Could you check a few things on this drawing? It's one solid part, dimensions in mm from its lowest x, y, z. A direction names the side the tool comes from. Coordinates: 2 decimals unless noted, no trailing zeros. Write each loop counter-clockwise with the first axis right and the second up, starting at its lowest first coordinate (ties: lowest second). Pieces come first, ordered by that corner, then holes.
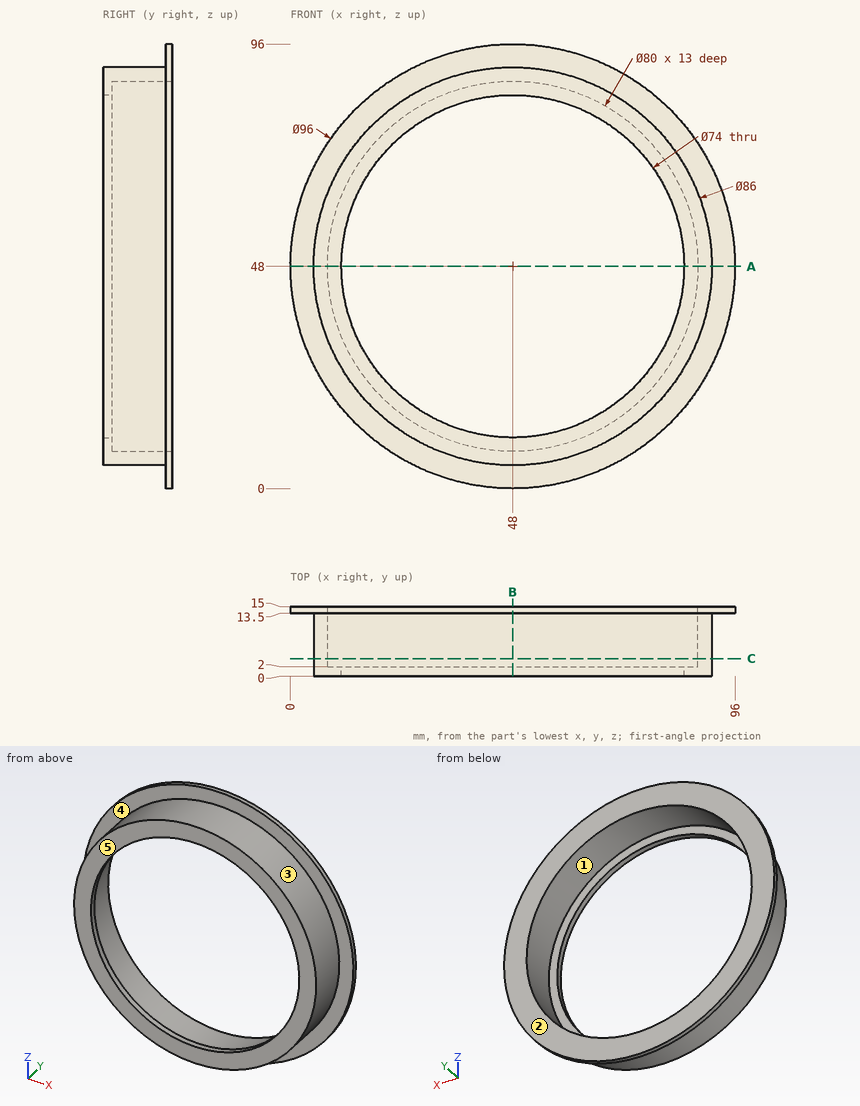
1) Imagine slicing it at B-B on x = 48. Please give me the cut outline in (y, z), then the cut area to 3 significant figures.
Values follow:
outline: (0, 5) - (13.5, 5) - (13.5, 0) - (15, 0) - (15, 8) - (2, 8) - (2, 11) - (0, 11) - close; (0, 85) - (2, 85) - (2, 88) - (15, 88) - (15, 96) - (13.5, 96) - (13.5, 91) - (0, 91) - close
area: 117 mm2
2) Imagine slicing it at A-A on z = 48. Please give me the cut outline in (x, y), then the cut area to 3 significant figures.
Values follow:
outline: (0, 13.5) - (5, 13.5) - (5, 0) - (11, 0) - (11, 2) - (8, 2) - (8, 15) - (0, 15) - close; (85, 0) - (91, 0) - (91, 13.5) - (96, 13.5) - (96, 15) - (88, 15) - (88, 2) - (85, 2) - close
area: 117 mm2
3) I need wall thicknesses on probe 1 along X at (y, z) = (9.75, 48); probe 2 along X at (y, z) = (1, 48); probe 3 along Z at (x, y) = (26, 10.25). Which ranges of each line are inside material? Lowest first, please.
Values follow:
probe 1: x = 5 to 8, 88 to 91
probe 2: x = 5 to 11, 85 to 91
probe 3: z = 11.05 to 14.59, 81.41 to 84.95
4) We'd pull the mould along X, two halves only. Please class the marked faces 1, 2 and 3: pulls with the +X half, pulls with the -X half, needs draft (parallel to the pull), parting line crosses it, or undercut.
Values follow:
face 1: undercut
face 2: needs draft
face 3: parting line crosses it
5) Imagine slicing it at C-C on y = 3.75. Please give me the cut outline in (x, z), then the cut area to 3 significant figures.
Values follow:
outline: circle Ø86 at (48, 48); hole circle Ø80 at (48, 48)
area: 782 mm2
6) On a 3-axis mill with a long thin cutter (end or side, diameter ignored), from which of +Z, -Z, +X, -X, +Y, -Y can I reach the whole of each face in a straight line? I mean the marked faces 4 and 5. Say none if no direction works.
Values follow:
face 4: -Y
face 5: +Z, -Z, +X, -X, -Y
7) Will these pins go through, and if not, where does the flat tip stop? pin 1 (4 mm diameter, centred on y = 9.5, z = 27.5, fed in from -X); pin 2 (8 mm diameter, centred on y = 2.5, z = 33.5, fed in from -X); pin 3 (1 mm diameter, centred on x = 86, y = 2.5, fed in from +Z); pin 4 (1 mm diameter, centred on x = 60, z = 14.5, fed in from +Y).
Values follow:
pin 1: stops at x = 9.18
pin 2: stops at x = 6.3
pin 3: stops at z = 69.04
pin 4: passes through
